Check sheet for the modelled part. Datum: model origin and axes. Units: mm. Face numbers are marked on the shaded views. Give positions to 0.01 mm unless a question says otherwise; leave off trailing zeros. Order: outer loops, then holes, each group sorted by start corner. A loop starts at its lowest first (then second) coordinate and runs counter-clockwise, first axis right, second up.
```python
from build123d import *
from OCP.BRepFilletAPI import BRepFilletAPI_MakeChamfer

# Parameters (mm, degrees)
SKETCH1_R        = 3.3235
BASENUT_DEPTH    = 4
ENDCHAMFER_SIZE  = 0.4
ENDCHAMFER_SIZE2 = 0.230940108


with BuildPart() as part:
    # Sketch1 → BaseNut (new body)
    with BuildSketch(Plane.XY):
        Polygon((3.75277675, -6.5), (7.505553499, 0), (3.75277675, 6.5), (-3.75277675, 6.5), (-7.505553499, 0), (-3.75277675, -6.5), align=None)
        Circle(SKETCH1_R, mode=Mode.SUBTRACT)
    extrude(amount=-BASENUT_DEPTH)

    # Sketch2 → Double-Chamfer (revolve, cut)
    with BuildSketch(Plane(origin=(0, 0, 0), x_dir=(1, 0, 0), z_dir=(0, 1, 0))):
        Polygon((-7.505553499, 4), (-6.125, 4), (-7.505553499, 3.202937065), align=None)
        Polygon((-7.505553499, 0.797062935), (-7.505553499, 0), (-6.125, 0), align=None)
    revolve(axis=Axis((0, 0, -3.375940562), (0, 0, 1)), mode=Mode.SUBTRACT)

    # EndChamfer: one chamfer whose edges measure the first distance from different faces: ONE call of the kernel's chamfer builder (chamfer() names one face for all edges)
    endchamfer_edges_1 = [part.edges().sort_by_distance(p)[0] for p in [
        (-3.3235, 0, -4),
    ]]
    endchamfer_side_1 = [part.faces().sort_by_distance(p)[0] for p in [
        (-3.3235, 0, -2),
    ]]
    endchamfer_edges_2 = [part.edges().sort_by_distance(p)[0] for p in [
        (-3.3235, 0, 0),
    ]]
    endchamfer_side_2 = [part.faces().sort_by_distance(p)[0] for p in [
        (5.951758839, 0, 0),
    ]]
    endchamfer = BRepFilletAPI_MakeChamfer(part.part.solid().wrapped)
    for e in endchamfer_edges_1:
        endchamfer.Add(ENDCHAMFER_SIZE, ENDCHAMFER_SIZE2, e.wrapped, endchamfer_side_1[0].wrapped)  # the first distance lies on this face
    for e in endchamfer_edges_2:
        endchamfer.Add(ENDCHAMFER_SIZE, ENDCHAMFER_SIZE2, e.wrapped, endchamfer_side_2[0].wrapped)  # the first distance lies on this face
    add(Compound.cast(endchamfer.Shape()), mode=Mode.REPLACE)


solid = part.part
```
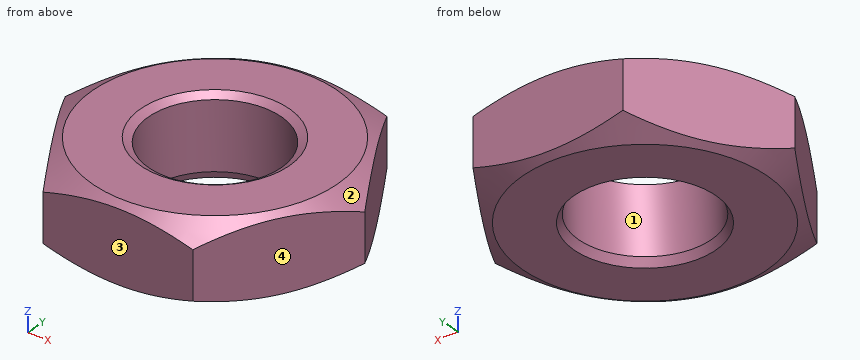
Q1. Material ranges on line 1 (Y direction, x = 0, z = -2.2); line 2 (X direction, y = 1.75, z = -3.35); line 3 (X direction, y = -1, z = -3.3), recorded low to high.
Q2. Sectioned sample at A-A, the plane x = 0. Record the cut outline in (y, z) (1 decimal), plus the area to 3 significant figures.
Q3. Go/stop test with flat-tipped pins: P1, Ø1, axis at y = 3, z = -3, coming from the +X side; P2, Ø4, axis at x = 0, y = 0, coming from the -Z side; P3, Ø1.5, axis at x = 2, y = 2.5, coming from the +Z side. Record where each tip stops, or that it passes through.
Q4. Draft check along X on the marked faces 1, 2, 3 and 4. Enter one of: pulls with the +X half, pulls with the -X half, needs draft (parallel to the pull), parting line crosses it, or undercut.
Q5. Sectioned sample at B-B, the plane z = -1.4. Record the cut outline in (x, y), plus the area to 3 significant figures.
Filled in:
1. line 1: y = -6.5 to -3.32, 3.32 to 6.5
1. line 2: x = -6.5 to -2.83, 2.83 to 6.5
1. line 3: x = -6.93 to -3.17, 3.17 to 6.93
2. outline: (-6.5, -3.8) - (-6.1, -4) - (-3.6, -4) - (-3.3, -3.6) - (-3.3, -0.2) - (-3.7, 0) - (-6.1, 0) - (-6.5, -0.2) - close; (3.3, -3.6) - (3.6, -4) - (6.1, -4) - (6.5, -3.8) - (6.5, -0.2) - (6.1, 0) - (3.7, 0) - (3.3, -0.2) - close
2. area: 25.1 mm2
3. P1: stops at x = 6.06
3. P2: passes through
3. P3: stops at z = 0
4. face 1: undercut
4. face 2: parting line crosses it
4. face 3: needs draft
4. face 4: pulls with the +X half
5. outline: (-7.51, 0) - (-3.75, -6.5) - (3.75, -6.5) - (7.51, 0) - (3.75, 6.5) - (-3.75, 6.5) - close; hole circle Ø6.65 at (0, 0)
5. area: 112 mm2
